from build123d import *

# Parameters (mm, degrees)
EXTRUDE_1_DEPTH         = 800
HOLE_WIZARD_3_5_3_5_1_D = 3.5


with BuildPart() as part:
    # 草图1 → 拉伸-薄壁1 (new body)
    with BuildSketch(Plane.XY):
        Polygon((0, 0), (8, 0), (8, 63), (0, 63), (0, 61.5), (6.5, 61.5), (6.5, 1.5), (0, 1.5), align=None)
    extrude(amount=EXTRUDE_1_DEPTH)

    # Ø3.5 (3.5) 直径孔1 (through all)
    with Locations(Plane(origin=(8, 0, 0), x_dir=(0, 0, -1), z_dir=(1, 0, 0))):
        with Locations((-775, 57.5), (-25, 57.5)):
            hole_wizard_3_5_3_5_1 = Hole(HOLE_WIZARD_3_5_3_5_1_D / 2)

    # 镜向1: Ø3.5 (3.5) 直径孔1 across plane
    add(hole_wizard_3_5_3_5_1.mirror(Plane(origin=(0, 31.5, 0), x_dir=(0, 0, 1), z_dir=(0, -1, 0))), mode=Mode.SUBTRACT)


solid = part.part
Read the model definition and answer for the solid it produces. Units are mm, in the model's axes. Coordinates: 2 decimals unless noted, no trailing zeros. Loops run counter-clockwise (first coordinate to the right, second up) from the corner with the lowest first, then second, coordinate; pieces in that order, holes last. Notation, with made-up numbers: (31.25, 63.25) - (39.25, 63.25) arc R20 cw to (39.25, 73.25) - close; hole circle Ø9 at (32.25, 62). An arc over 180 degrees is marked (long way). Answer in a Markdown table with one row per item.
Q1. Find section B-B on z = 551. Write down the section's boundary in (x, y).
Here are the results:
| item | result |
|---|---|
| outline | (0, 0) - (8, 0) - (8, 63) - (0, 63) - (0, 61.5) - (6.5, 61.5) - (6.5, 1.5) - (0, 1.5) - close |
Q2. Find section C-C on y = 39.5. Write down the section's boundary in (x, z), plus the area to 3 significant figures.
Here are the results:
| item | result |
|---|---|
| outline | (6.5, 0) - (8, 0) - (8, 800) - (6.5, 800) - close |
| area | 1,200 mm^2 |
Q3. The mould has two halves that part along Y. Classify faces 1 (the flat face through (6.5, 32, 394)), 2 (the flat face through (8, 31, 394)): pulls with the +Y half, pulls with the -Y half, needs draft (parallel to the pull), parting line crosses it, or undercut.
Here are the results:
| item | result |
|---|---|
| face 1 | undercut |
| face 2 | needs draft |
Q4. Straight lines are drawn through the part: line 1 along Y through (x, z) = (7.2, 775); line 2 along Y through (x, z) = (0.5, 576); line 3 along X through (y, z) = (32, 568.5). For each, find the intervals that lie inside material, in ascending order. Write a range as [from, to].
Here are the results:
| item | result |
|---|---|
| line 1 | y = [0, 3.75], [7.25, 55.75], [59.25, 63] |
| line 2 | y = [0, 1.5], [61.5, 63] |
| line 3 | x = [6.5, 8] |
Q5. Given P1, Ø4, axis at y = 57.5, z = 775, coming from the -X side; P2, Ø1.5, axis at x = 4.5, z = 718, coming from the -Y side, each flat-ended and moving along its own axis, determine where each tip first touches the part or whether it passes through.
Here are the results:
| item | result |
|---|---|
| P1 | stops at x = 6.5 |
| P2 | stops at y = 0 |
Q6. Find section A-A on x = 3.75. Write down the section's boundary in (y, z).
Here are the results:
| item | result |
|---|---|
| outline | (0, 0) - (1.5, 0) - (1.5, 800) - (0, 800) - close; (61.5, 0) - (63, 0) - (63, 800) - (61.5, 800) - close |
